Read the model definition and answer for the solid it produces. Units are mm, in the model's axes. Face numbers are marked on the shaded views. A direction names the side the tool comes from. Coordinates: 2 decimals unless noted, no trailing zeros. Order: outer loops, then holes, each group sorted by start corner. A loop starts at its lowest first (then second) coordinate and runs counter-clockwise, first axis right, second up.
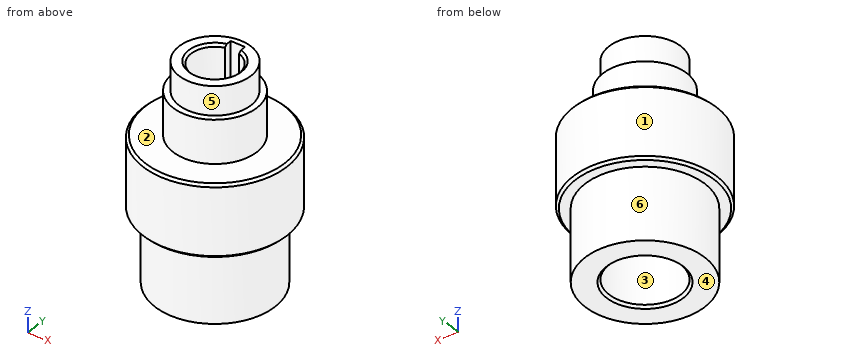
```python
from build123d import *

# Parameters (mm, degrees)
SKETCH_1_R          = 25
EXTRUDE_1_DEPTH     = 30
SKETCH_2_R          = 30
EXTRUDE_2_DEPTH     = 40
SKETCH_4_R          = 10
CUT_EXTRUDE_1_DEPTH = 82.853527719
SKETCH_11_W         = 6
SKETCH_11_H         = 3.260607986
CUT_EXTRUDE_3_DEPTH = 82.853527719
SKETCH_12_R         = 15
CUT_EXTRUDE_4_DEPTH = 30
SKETCH_13_R         = 17.5
EXTRUDE_4_DEPTH     = 20
CUT_EXTRUDE_START   = -10
SKETCH_14_R         = 30
SKETCH_14_R_2       = 17.5
CUT_EXTRUDE_5_DEPTH = 10
CUT_EXTRUDE_START_2 = -12
SKETCH_15_R         = 17.5
SKETCH_15_R_2       = 15
CUT_EXTRUDE_6_DEPTH = 12
CHAMFER_2_SIZE      = 1


with BuildPart() as part:
    # 草图1 → 凸台-拉伸1 (new body)
    with BuildSketch(Plane.XY):
        Circle(SKETCH_1_R)
    extrude(amount=EXTRUDE_1_DEPTH)

    # 草图2 → 凸台-拉伸2 (add)
    with BuildSketch(Plane.XY.offset(30)):
        Circle(SKETCH_2_R)
    extrude(amount=EXTRUDE_2_DEPTH)

    # 草图4 → 切除-拉伸1 (cut, through all)
    with BuildSketch(Plane(origin=(0, 0, 0), x_dir=(-1, 0, 0), z_dir=(0, 0, -1))):
        Circle(SKETCH_4_R)
    extrude(amount=-CUT_EXTRUDE_1_DEPTH, mode=Mode.SUBTRACT)

    # 草图11 → 切除-拉伸3 (cut, through all)
    with BuildSketch(Plane.XY.offset(70)):
        with Locations((0, 11.169696007)):
            Rectangle(SKETCH_11_W, SKETCH_11_H)
    extrude(amount=-CUT_EXTRUDE_3_DEPTH, mode=Mode.SUBTRACT)

    # 草图12 → 切除-拉伸4 (cut)
    with BuildSketch(Plane(origin=(0, 0, 0), x_dir=(-1, 0, 0), z_dir=(0, 0, -1))):
        Circle(SKETCH_12_R)
    extrude(amount=-CUT_EXTRUDE_4_DEPTH, mode=Mode.SUBTRACT)

    # 草图13 → 凸台-拉伸4 (add)
    with BuildSketch(Plane.XY.offset(70)):
        Circle(SKETCH_13_R)
        with BuildLine():
            Line((3, 9.539392014), (3, 12.8))
            Line((3, 12.8), (-3, 12.8))
            Line((-3, 12.8), (-3, 9.539392014))
            ThreePointArc((-3, 9.539392014), (0, -10), (3, 9.539392014))
        make_face(mode=Mode.SUBTRACT)
    extrude(amount=EXTRUDE_4_DEPTH)

    # 草图14 → 切除-拉伸5 (cut)
    with BuildSketch(Plane.XY.offset(70).offset(CUT_EXTRUDE_START)):
        Circle(SKETCH_14_R)
        Circle(SKETCH_14_R_2, mode=Mode.SUBTRACT)
    extrude(amount=CUT_EXTRUDE_5_DEPTH, mode=Mode.SUBTRACT)

    # 草图15 → 切除-拉伸6 (cut)
    with BuildSketch(Plane.XY.offset(90).offset(CUT_EXTRUDE_START_2)):
        Circle(SKETCH_15_R)
        with Locations(Location((0, 0, 0), (0, 0, 180))):
            Circle(SKETCH_15_R_2, mode=Mode.SUBTRACT)
    extrude(amount=CUT_EXTRUDE_6_DEPTH, mode=Mode.SUBTRACT)

    # 倒角2
    chamfer_2_edges = [part.edges().sort_by_distance(p)[0] for p in [
        (15, 0, 0),
        (0, -10, 90),
        (-30, 0, 30),
        (-30, 0, 60),
    ]]
    chamfer(chamfer_2_edges, length=CHAMFER_2_SIZE)


solid = part.part
```
1) Which of the six approach directions +Z, -Z, +X, -X, +Y, -Y give full straight-line access (tool end or side, diameter ignored) to the marked faces 4, 5 and 6?
A:
face 4: -Z, +X, -X, +Y, -Y
face 5: +Z
face 6: -Z
2) A cutting plane is placed at D-D, the plane z = 22.5. Determine the outline of the cut face in (x, y).
A:
outline: circle Ø50 at (0, 0); hole circle Ø30 at (0, 0)
3) Determine the mould class of the marked faces 1, 2 and 3 for opening direction X: pulls with the +X half, pulls with the -X half, needs draft (parallel to the pull), parting line crosses it, or undercut.
A:
face 1: parting line crosses it
face 2: needs draft
face 3: undercut
4) Straight lines are drawn through the part: line 1 (Y direction, x = 0, z = 39.5); line 2 (Y direction, x = 0, z = 24.25); line 3 (Z direction, x = 14.5, y = -8). For each, find the intervals that lie inside material, in ascending order.
A:
line 1: y = -30 to -10, 12.8 to 30
line 2: y = -25 to -15, 15 to 25
line 3: z = 0 to 78
5) Flat-ended cylindrical pins translate along their axes: pin 1 Ø3 at (x, z) = (-1, 51) entering from -Y; pin 2 Ø3.5 at (y, z) = (10.5, 57.5) entering from -X; pin 3 Ø4 at (x, z) = (2.5, 53.5) entering from +Y; pin 4 Ø17.5 at (x, y) = (1.5, 9.5) entering from -Z. Find the tip coordinate at first contact, or state that the pin passes through.
A:
pin 1: stops at y = -30
pin 2: stops at x = -28.7
pin 3: stops at y = 30
pin 4: stops at z = 0
6) A cutting plane is placed at C-C, the plane z = 74. Determine the outline of the cut face in (x, y).
A:
outline: circle Ø35 at (0, 0); hole (-3, 9.54) arc R10 ccw (long way) to (3, 9.54) - (3, 12.8) - (-3, 12.8) - close
